Answer from the drawing. Dimensions are ordinates in mm from the lowest x, y and z of the part. Coordinates: 2 decimals unless noted, no trailing zeros. Write each loop counter-clockwise with the first axis right and the second up, starting at its lowest first coordinate (ties: lowest second). Pieces come first, ordered by that corner, then holes. Notation, with made-up numbers: (28.5, 34.25) -> (69.5, 34.25) arc R38 ccw to (69.5, 73.25) -> close; hole circle Ø3 at (-4, 50.5). An arc over 180 degrees is marked (long way). Answer as a JSON object with one key per item and string values. Group by question number.
(1) For a pull along X with two mould halves and no side action, classify the marked faces 1, 2 and 3 as +X half, -X half, draft (parallel to the pull), parting line (faces both ways), or undercut.
(2) Find section A-A (x = 42.5). Give the vertices of the cut face in (y, z).
(3) Find section B-B (y = 25). Give the vertices of the cut face in (x, z), then the cut area to 3 significant figures.
(4) Straight lines are drawn through the part: L1, parallel to Y at x = 42.5, z = 3.1; L2, parallel to X at y = 25.5, z = 1; L3, parallel to X at y = 30.5, z = 1.3. For each, find the intervals that lie inside material, in ascending order.
(5) Find section C-C (z = 5.05). Give the vertices of the cut face in (x, y), then the cut area to 3 significant figures.
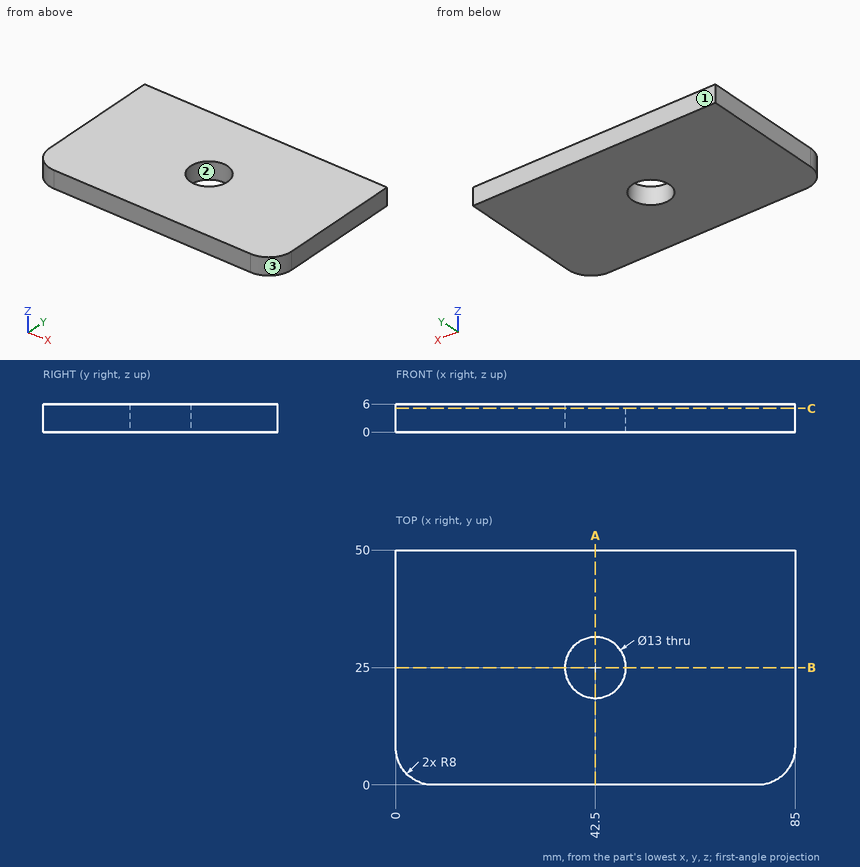
Results below:
{
 "1": {"face 1": "draft", "face 2": "undercut", "face 3": "+X half"},
 "2": {"outline": "(0, 0) -> (18.5, 0) -> (18.5, 6) -> (0, 6) -> close; (31.5, 0) -> (50, 0) -> (50, 6) -> (31.5, 6) -> close"},
 "3": {"outline": "(0, 0) -> (36, 0) -> (36, 6) -> (0, 6) -> close; (49, 0) -> (85, 0) -> (85, 6) -> (49, 6) -> close", "area": "432 mm2"},
 "4": {"L1": "y = 0 to 18.5, 31.5 to 50", "L2": "x = 0 to 36.02, 48.98 to 85", "L3": "x = 0 to 39.04, 45.96 to 85"},
 "5": {"outline": "(0, 8) arc R8 ccw to (8, 0) -> (77, 0) arc R8 ccw to (85, 8) -> (85, 50) -> (0, 50) -> close; hole circle Ø13 at (42.5, 25)", "area": "4,090 mm2"}
}
